from build123d import *

# Parameters (mm, degrees)
BASE_BLOCK_DEPTH           = 10
LUG_TAB_PROFILE_W          = 40
LUG_TAB_PROFILE_H          = 40
LUG_TAB_DEPTH              = 5
LUG_TAB_EDGE_FILLET_RADIUS = 20
LUG_TAB_EDGE_FILLET_LENGTH = 10
CORNER_FILLET_R10_R        = 10
CROSS_HOLE_PROFILE_R       = 10
CROSS_HOLE_20_DEPTH        = 72.589105316
LUG_HOLE_PROFILE_R         = 10
LUG_HOLE_20_DEPTH          = 71


with BuildPart() as part:
    # Base Block Profile → Base Block (new, symmetric)
    with BuildSketch(Plane.XY):
        with BuildLine():
            Line((20, -25), (-10, -25))
            ThreePointArc((-10, -25), (-17.071067812, -22.071067812), (-20, -15))
            Line((-20, -15), (-20, 15))
            ThreePointArc((-20, 15), (-17.071067812, 22.071067812), (-10, 25))
            Line((-10, 25), (20, 25))
            Line((20, 25), (20, -25))
        make_face()
    extrude(amount=BASE_BLOCK_DEPTH, both=True)

    # Lug Tab Profile → Lug Tab (add, symmetric)
    with BuildSketch(Plane(origin=(0, 0, 0), x_dir=(1, 0, 0), z_dir=(0, 1, 0))):
        with Locations((40, 0)):
            Rectangle(LUG_TAB_PROFILE_W, LUG_TAB_PROFILE_H)
    extrude(amount=LUG_TAB_DEPTH, both=True)

    # Lug Tab Edge Fillet: full round fillet: the end face becomes a half cylinder, R = half its width
    lug_tab_edge_fillet_face = Plane((60, 0, 0), x_dir=(0, -1, 0), z_dir=(1, 0, 0))  # on the end face: x along it, z out of the body
    lug_tab_edge_fillet_slab = lug_tab_edge_fillet_face.offset(-LUG_TAB_EDGE_FILLET_RADIUS / 2) * Box(LUG_TAB_EDGE_FILLET_LENGTH, 2 * LUG_TAB_EDGE_FILLET_RADIUS, LUG_TAB_EDGE_FILLET_RADIUS, mode=Mode.PRIVATE)  # the body's end, R deep
    lug_tab_edge_fillet_round = Plane((40, 0, 0), x_dir=(1, 0, 0), z_dir=(0, -1, 0)) * Cylinder(LUG_TAB_EDGE_FILLET_RADIUS, LUG_TAB_EDGE_FILLET_LENGTH, mode=Mode.PRIVATE)  # its axis R under the face
    add(lug_tab_edge_fillet_slab - lug_tab_edge_fillet_round, mode=Mode.SUBTRACT)

    # Corner Fillet R10
    corner_fillet_r10_edges = [part.edges().sort_by_distance(p)[0] for p in [
        (20, 5, 0),
        (20, -5, 0),
    ]]
    fillet(corner_fillet_r10_edges, radius=CORNER_FILLET_R10_R)

    # Cross Hole Profile → Cross Hole _20 (cut, through all)
    with BuildSketch(Plane.XY.offset(10)):
        with Locations((0, 5)):
            Circle(CROSS_HOLE_PROFILE_R)
    extrude(amount=-CROSS_HOLE_20_DEPTH, mode=Mode.SUBTRACT)

    # Lug Hole Profile → Lug Hole _20 (cut, through all)
    with BuildSketch(Plane(origin=(0, 5, 0), x_dir=(1, 0, 0), z_dir=(0, 1, 0))):
        with Locations(Location((40, 0, 0), (0, 0, 180))):
            Circle(LUG_HOLE_PROFILE_R)
    extrude(amount=-LUG_HOLE_20_DEPTH, mode=Mode.SUBTRACT)


solid = part.part
Here's how the part is built. I have some questions about the finished solid (model axes, mm). A direction names the side the tool comes from. Give positions to 0.01 mm unless a question says otherwise; leave off trailing zeros. Loops run counter-clockwise (first coordinate to the right, second up) from the corner with the lowest first, then second, coordinate; pieces in that order, holes last. Notation, with made-up numbers: (20.25, 84) -> (57.25, 84) arc R8 cw to (57.25, 96) -> close; hole circle Ø2 at (33.5, 35.5). An arc over 180 degrees is marked (long way). Answer as a JSON object with one key per item and string values. Group by question number.
Item 1: I need wall thicknesses on L1, parallel to Y at x = 0, z = -4.25; L2, parallel to Z at x = 40, y = -0.5; L3, parallel to Y at x = 31, z = -11. Which ranges of each line are inside material? Lowest first, please.
Item 2: On a 3-axis mill with a long thin cutter (end or side, diameter ignored), from which of +Z, -Z, +X, -X, +Y, -Y can I reach the whole of each face in a straight line? I mean faces 5 (the flat face through (20, -20, 0)), 6 (the flat face through (20, 0, 15)), 7 (the flat face through (20, 0, -15)), 8 (the flat face through (20, 20, 0)). Say none if no direction works.
Item 3: Will these pins go through, and if not, where does the flat tip stop? pin 1 (2 mm diameter, centred on x = 24, z = 15, fed in from +Y); pin 2 (3 mm diameter, centred on y = -20.5, z = -4, fed in from +X); pin 3 (3 mm diameter, centred on x = 12.5, y = 16.5, fed in from +Z).
Item 4: Imagine slicing it at D-D on y = 11.5. Write out the boundary of the cut face in (x, z).
Item 5: Imagine slicing it at B-B on z = -7.5. Write out the boundary of the cut face in (x, y), then the cut area to 3 significant figures.
Item 6: Imagine slicing it at A-A on x = 0. Write out the boundary of the cut face in (y, z), then the cut area to 3 significant figures.
Item 7: Thinking about a two-plate mould opening in Y: for faces 1 (the flat face through (5, -25, 0)), 2 (the cylindrical face through (-1.302, 14.915, 0.14)), 3 (the cylindrical face through (22.85, 8.01, -0.14)), 4 (the flat face through (-0.2, -5.2, -10)), which applies, pulls with the +Y half, pulls with the -Y half, needs draft (parallel to the pull), parting line crosses it, or undercut?
Item 8: Imagine slicing it at C-C on y = 1. Write out the boundary of the cut face in (x, z).
Answer list:
{
 "1": {"L1": "y = -25 to -5, 15 to 25", "L2": "z = -20 to -10, 10 to 20", "L3": "y = -5 to 5"},
 "2": {"face 5": "+Z, -Z, +X, -Y", "face 6": "+Z, -X, +Y, -Y", "face 7": "-Z, -X, +Y, -Y", "face 8": "+Z, -Z, +X, +Y"},
 "3": {"pin 1": "stops at y = 5", "pin 2": "stops at x = 20", "pin 3": "stops at z = 10"},
 "4": {"outline": "(-20, -10) -> (-7.6, -10) -> (-7.6, 10) -> (-20, 10) -> close; (7.6, -10) -> (20.63, -10) -> (20.63, 10) -> (7.6, 10) -> close"},
 "5": {"outline": "(-20, -15) arc R10 ccw to (-10, -25) -> (20, -25) -> (20, -15) arc R10 cw to (30, -5) -> (33.39, -5) -> (33.39, 5) -> (30, 5) arc R10 cw to (20, 15) -> (20, 25) -> (-10, 25) arc R10 ccw to (-20, 15) -> close; (46.61, -5) -> (58.54, -5) -> (58.54, 5) -> (46.61, 5) -> close; hole circle Ø20 at (0, 5)", "area": "1,940 mm2"},
 "6": {"outline": "(-25, -10) -> (-5, -10) -> (-5, 10) -> (-25, 10) -> close; (15, -10) -> (25, -10) -> (25, 10) -> (15, 10) -> close", "area": "600 mm2"},
 "7": {"face 1": "pulls with the -Y half", "face 2": "undercut", "face 3": "pulls with the +Y half", "face 4": "needs draft"},
 "8": {"outline": "(-20, -10) -> (-9.17, -10) -> (-9.17, 10) -> (-20, 10) -> close; (9.17, -10) -> (20, -10) -> (20, -20) -> (40, -20) arc R20 ccw to (40, 20) -> (20, 20) -> (20, 10) -> (9.17, 10) -> close; hole circle Ø20 at (40, 0)"}
}
